```python
from build123d import *

# Parameters (mm, degrees)
SKETCH1_W           = 160
SKETCH1_H           = 220
BOSS_EXTRUDE1_DEPTH = 1000
SKETCH2_R           = 19
CUT_EXTRUDE1_DEPTH  = 30


with BuildPart() as part:
    # Sketch1 → Boss-Extrude1 (new body)
    with BuildSketch(Plane.XY):
        Polygon((-290, 260), (290, 260), (290, 240), (100, 240), (100, 20), (290, 20), (290, 0), (-290, 0), (-290, 20), (-100, 20), (-100, 240), (-290, 240), align=None)
        with Locations((0, 130)):
            Rectangle(SKETCH1_W, SKETCH1_H, mode=Mode.SUBTRACT)
    extrude(amount=BOSS_EXTRUDE1_DEPTH)

    # Sketch2 → Cut-Extrude1 (cut)
    with BuildSketch(Plane(origin=(0, 0, 0), x_dir=(-1, 0, 0), z_dir=(0, -1, 0))):
        with Locations(Location((205.124206689, -955.639521656, 0), (0, 0, 90))):
            Circle(SKETCH2_R)
        with Locations(Location((-205.124206689, -955.639521656, 0), (0, 0, 90))):
            Circle(SKETCH2_R)
        with Locations(Location((-205.124206689, -44.360478344, 0), (0, 0, 90))):
            Circle(SKETCH2_R)
        with Locations(Location((205.124206689, -44.360478344, 0), (0, 0, 90))):
            Circle(SKETCH2_R)
    extrude(amount=-CUT_EXTRUDE1_DEPTH, mode=Mode.SUBTRACT)


solid = part.part
```
CAD build for the part. Positions are in the model's coordinates, mm. A direction names the side the tool comes from. Round coordinates to 2 decimals unless told otherwise and drop trailing zeros. Write each loop counter-clockwise with the first axis right and the second up, starting at its lowest first coordinate (ties: lowest second). Pieces come first, ordered by that corner, then holes. Notation, with made-up numbers: (-10.75, -27) - (-6.75, -27) arc R5 ccw to (-6.75, -21) - close; hole circle Ø4 at (-16, 7). An arc over 180 degrees is marked (long way). Return JSON: item names as keys, results as strings. Group by question number.
Item 1: Flat gauge pins, fed straight in: pin 1 Ø4 at (y, z) = (204, 839.5) entering from -X; pin 2 Ø12 at (y, z) = (138.5, 458) entering from +X. Where does each tip first touch, or does it go through?
Item 2: Band-saw the part on C-C on z = 137.5. List the corners of the cut face in (x, y), plus the area to 3 significant figures.
Item 3: Band-saw the part on B-B on y = 169. List the corners of the cut face in (x, z), plus the area to 3 significant figures.
Item 4: Probe probe 1 along Y at (x, z) = (-61, 368.5); probe 2 along X at (y, z) = (211, 363). List the from-to ranges inside material, lowest first.
Item 5: Band-saw the part on A-A on x = -110.5. List the corners of the cut face in (y, z).
Item 6: 3-axis set-ups, long thin cutter, end or side, ignore diameter. For faces 1 (the face through (-196, 20, 493)), 2 (the face through (-1, 240, 493)), 3 (the face through (205.96, 9.86, 974.62)), 4 (the face through (100, 132, 493)): which of +Z, -Z, +X, -X, +Y, -Y reach the whole face in a straight line?
Item 7: Mould opens along Z. For faces 5 (the face through (290, 10, 493)), 6 (the face through (87, 121, 1000)), 7 (the face through (205.96, 9.86, 63.342)), 8 (the face through (-223.672, 9.86, 48.479)) say: +Z half, -Z half, draft (parallel to the pull), parting line (faces both ways), or undercut.
Resolved:
{
 "1": {"pin 1": "stops at x = -100", "pin 2": "stops at x = 100"},
 "2": {"outline": "(-290, 0) - (290, 0) - (290, 20) - (100, 20) - (100, 240) - (290, 240) - (290, 260) - (-290, 260) - (-290, 240) - (-100, 240) - (-100, 20) - (-290, 20) - close; hole (-80, 20) - (80, 20) - (80, 240) - (-80, 240) - close", "area": "32,000 mm²"},
 "3": {"outline": "(-100, 0) - (-80, 0) - (-80, 1000) - (-100, 1000) - close; (80, 0) - (100, 0) - (100, 1000) - (80, 1000) - close", "area": "40,000 mm²"},
 "4": {"probe 1": "y = 0 to 20, 240 to 260", "probe 2": "x = -100 to -80, 80 to 100"},
 "5": {"outline": "(0, 0) - (20, 0) - (20, 1000) - (0, 1000) - close; (240, 0) - (260, 0) - (260, 1000) - (240, 1000) - close"},
 "6": {"face 1": "+Z, -Z, -X", "face 2": "+Z, -Z", "face 3": "-Y", "face 4": "+Z, -Z, +X"},
 "7": {"face 5": "draft", "face 6": "+Z half", "face 7": "undercut", "face 8": "undercut"}
}
